```python
from build123d import *

# Parameters (mm, degrees)
EXTRUDE_1_DEPTH        = 18
CHAMFER_1_SIZE         = 2
HOLE_WIZARD_M4_1_D     = 3.3
HOLE_WIZARD_M4_1_DEPTH = 10.1
HOLE_WIZARD_M4_1_TIP   = 0.991420021
HOLE_WIZARD_M5_1_D     = 4.2
HOLE_WIZARD_M5_1_DEPTH = 12.4
HOLE_WIZARD_M5_1_TIP   = 1.2618073


with BuildPart() as part:
    # 草图1 → 拉伸-薄壁1 (new, symmetric)
    with BuildSketch(Plane.XY):
        Polygon((0, 0), (0, 37.5), (30, 37.5), (30, 27.5), (10, 27.5), (10, 0), align=None)
    extrude(amount=EXTRUDE_1_DEPTH, both=True)

    # 倒角1
    chamfer_1_edges = [part.edges().sort_by_distance(p)[0] for p in [
        (5, 0, 18),
        (5, 0, -18),
        (30, 32.5, -18),
        (30, 32.5, 18),
    ]]
    chamfer(chamfer_1_edges, length=CHAMFER_1_SIZE)

    # M4 螺纹孔1
    with Locations(Plane.ZY):
        with Locations((12.5, 27), (12.5, 6), (-12.5, 6), (-12.5, 27)):
            Hole(HOLE_WIZARD_M4_1_D / 2, depth=HOLE_WIZARD_M4_1_DEPTH)
            with Locations((0, 0, -(HOLE_WIZARD_M4_1_DEPTH + HOLE_WIZARD_M4_1_TIP / 2))):  # 118° drill point
                Cone(0, HOLE_WIZARD_M4_1_D / 2, HOLE_WIZARD_M4_1_TIP, mode=Mode.SUBTRACT)

    # M5 螺纹孔1
    with Locations(Plane(origin=(0, 27.5, 0), x_dir=(-1, 0, 0), z_dir=(0, -1, 0))):
        with Locations((-20, 12.5), (-20, -12.5)):
            Hole(HOLE_WIZARD_M5_1_D / 2, depth=HOLE_WIZARD_M5_1_DEPTH)
            with Locations((0, 0, -(HOLE_WIZARD_M5_1_DEPTH + HOLE_WIZARD_M5_1_TIP / 2))):  # 118° drill point
                Cone(0, HOLE_WIZARD_M5_1_D / 2, HOLE_WIZARD_M5_1_TIP, mode=Mode.SUBTRACT)


solid = part.part
```
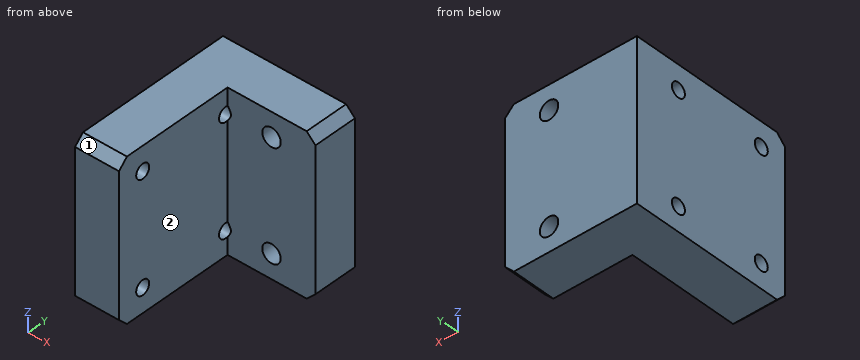
Here's how the part is built. I have some questions about the finished solid (model axes, mm). Face numbers are marked on the shaded views. A direction names the side the tool comes from. Give positions to 0.01 mm unless a question says otherwise; leave off trailing zeros. Order: outer loops, then holes, each group sorted by start corner. A loop starts at its lowest first (then second) coordinate and runs counter-clockwise, first axis right, second up. Notation, with made-up numbers: (79.5, 69) - (83.5, 69) arc R30 ccw to (83.5, 108) - close; hole circle Ø7 at (81.5, 17). An arc over 180 degrees is marked (long way). Answer as a JSON object with one key per item and string values. Group by question number.
Item 1: For P1, Ø10, axis at x = 16.5, z = 7, coming from the -Y side; P2, Ø14, axis at y = 10.5, z = -3.5, coming from the +X side; P3, Ø3, axis at y = 27, z = -12.5, coming from the -X side, each with a flat end and sliding along its axis, tell me the tip position at first contact or that it passes through.
Item 2: Please list where these lines run through material, in increasing order: probe 1 along Z at (x, y) = (20, 30.75); probe 2 along X at (y, z) = (30.5, 12.5); probe 3 along X at (y, z) = (22, -8).
Item 3: If we section it at C-C on x = 6.5: Please give me the cut outline in (y, z).
Item 4: If we section it at B-B on y = 6: Please give me the cut outline in (x, z).
Item 5: Which directions (+Z, -Z, +X, -X, +Y, -Y) give clear straight access to the entire face, cutting with the end or side of a thin tool? Please do the marked faces 1 and 2.
Item 6: If we section it at D-D on x = 18.5: Please give me the cut outline in (y, z), and give its area (3 significant figures).
Item 7: If we section it at A-A on z = -12.5: Please give me the cut outline in (x, y).
Result set:
{
 "1": {"P1": "y = 27.5", "P2": "x = 10", "P3": "x = 10.19"},
 "2": {"probe 1": "-18 to -14.6, -10.4 to 10.4, 14.6 to 18", "probe 2": "0 to 17.9, 22.1 to 30", "probe 3": "0 to 10"},
 "3": {"outline": "(0, -16) - (2, -18) - (37.5, -18) - (37.5, 18) - (2, 18) - (0, 16) - close; hole circle Ø3.3 at (6, -12.5); hole circle Ø3.3 at (6, 12.5); hole circle Ø3.3 at (27, -12.5); hole circle Ø3.3 at (27, 12.5)"},
 "4": {"outline": "(0, -18) - (10, -18) - (10, -14.15) - (0, -14.15) - close; (0, -10.85) - (10, -10.85) - (10, 10.85) - (0, 10.85) - close; (0, 14.15) - (10, 14.15) - (10, 18) - (0, 18) - close"},
 "5": {"face 1": "+Z, +X, -X, -Y", "face 2": "+Z, -Z, +X, -Y"},
 "6": {"outline": "(27.5, -18) - (37.5, -18) - (37.5, -13.97) - (27.5, -13.97) - close; (27.5, -11.03) - (37.5, -11.03) - (37.5, 11.03) - (27.5, 11.03) - close; (27.5, 13.97) - (37.5, 13.97) - (37.5, 18) - (27.5, 18) - close", "area": "301 mm²"},
 "7": {"outline": "(0, 0) - (10, 0) - (10, 4.35) - (0, 4.35) - close; (0, 7.65) - (10, 7.65) - (10, 25.35) - (0, 25.35) - close; (0, 28.65) - (10.1, 28.65) - (10.79, 27.5) - (17.9, 27.5) - (17.9, 37.5) - (0, 37.5) - close; (22.1, 27.5) - (30, 27.5) - (30, 37.5) - (22.1, 37.5) - close"}
}
